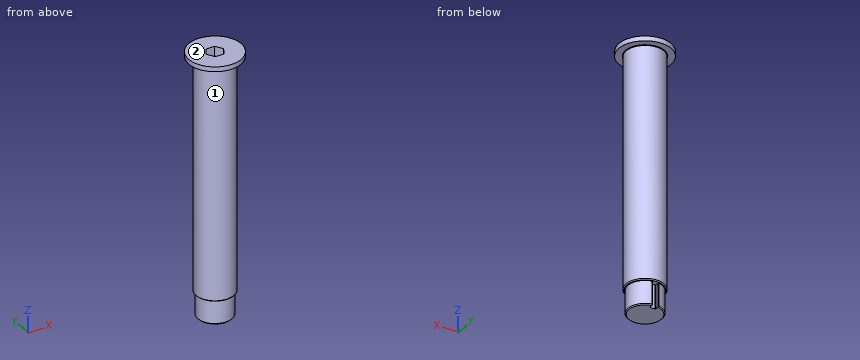
```python
from build123d import *

# Parameters (mm, degrees)
SKETCH_1_R          = 20
EXTRUDE_1_DEPTH     = 270
SKETCH_2_R          = 27.5
EXTRUDE_2_DEPTH     = 5
CUT_EXTRUDE_1_DEPTH = 10
SKETCH_4_OUTSIDE_W  = 114.158
SKETCH_4_OUTSIDE_H  = 114.158
SKETCH_4_OUTSIDE_R  = 18
CUT_EXTRUDE_2_DEPTH = 25
CHAMFER_1_SIZE      = 1
CHAMFER_2_SIZE      = 1
FILLET_1_R          = 0.5
SKETCH_5_W          = 6
SKETCH_5_H          = 10
CUT_EXTRUDE_3_DEPTH = 25
FILLET_2_R          = 0.5


with BuildPart() as part:
    # 草图1 → 凸台-拉伸1 (new body)
    with BuildSketch(Plane.XY):
        Circle(SKETCH_1_R)
    extrude(amount=EXTRUDE_1_DEPTH)

    # 草图2 → 凸台-拉伸2 (add)
    with BuildSketch(Plane.XY.offset(270)):
        Circle(SKETCH_2_R)
    extrude(amount=EXTRUDE_2_DEPTH)

    # 草图3 → 切除-拉伸1 (cut)
    with BuildSketch(Plane.XY.offset(275)):
        Polygon((9.237604307, 0), (4.618802154, 8), (-4.618802154, 8), (-9.237604307, 0), (-4.618802154, -8), (4.618802154, -8), align=None)
    extrude(amount=-CUT_EXTRUDE_1_DEPTH, mode=Mode.SUBTRACT)

    # 草图4 outside → 切除-拉伸2 (cut)
    with BuildSketch(Plane(origin=(0, 0, 0), x_dir=(-1, 0, 0), z_dir=(0, 0, -1))):
        Rectangle(SKETCH_4_OUTSIDE_W, SKETCH_4_OUTSIDE_H)
        Circle(SKETCH_4_OUTSIDE_R, mode=Mode.SUBTRACT)
    extrude(amount=-CUT_EXTRUDE_2_DEPTH, mode=Mode.SUBTRACT)

    # 倒角1
    chamfer_1_edges = [part.edges().sort_by_distance(p)[0] for p in [
        (-20, 0, 25),
    ]]
    chamfer(chamfer_1_edges, length=CHAMFER_1_SIZE)

    # 倒角2
    chamfer_2_edges = [part.edges().sort_by_distance(p)[0] for p in [
        (18, 0, 0),
    ]]
    chamfer(chamfer_2_edges, length=CHAMFER_2_SIZE)

    # 圆角1
    fillet_1_edges = [part.edges().sort_by_distance(p)[0] for p in [
        (-20, 0, 270),
    ]]
    fillet(fillet_1_edges, radius=FILLET_1_R)

    # 草图5 → 切除-拉伸3 (cut)
    with BuildSketch(Plane(origin=(0, 0, 0), x_dir=(-1, 0, 0), z_dir=(0, 0, -1))):
        with Locations((0, 18)):
            Rectangle(SKETCH_5_W, SKETCH_5_H)
    extrude(amount=-CUT_EXTRUDE_3_DEPTH, mode=Mode.SUBTRACT)

    # 圆角2
    fillet_2_edges = [part.edges().sort_by_distance(p)[0] for p in [
        (3, 13, 12.5),
        (-3, 13, 12.5),
        (-3, 17.748239349, 13),
        (3, 17.748239349, 13),
    ]]
    fillet(fillet_2_edges, radius=FILLET_2_R)


solid = part.part
```
The listing builds one solid part. Answer for the finished solid, in the listing's coordinates (mm). Face numbers are marked on the shaded views. A direction names the side the tool comes from. Give positions to 0.01 mm unless a question says otherwise; leave off trailing zeros. Order: outer loops, then holes, each group sorted by start corner. A loop starts at its lowest first (then second) coordinate and runs counter-clockwise, first axis right, second up.
Item 1: The part is cut by section B-B, the plane z = 235. Give the vertices of the cut face in (x, y), and give its area (3 significant figures).
From the geometry:
outline: circle Ø40 at (0, 0)
area: 1,260 mm2
Item 2: The part is cut by section A-A, the plane x = 0. Give the vertices of the cut face in (y, z), and give its area (3 significant figures).
From the geometry:
outline: (-27.5, 270) - (-20.5, 270) arc R0.5 cw to (-20, 269.5) - (-20, 26) - (-19, 25) - (-18, 25) - (-18, 1) - (-17, 0) - (13, 0) - (13, 25) - (19, 25) - (20, 26) - (20, 269.5) arc R0.5 cw to (20.5, 270) - (27.5, 270) - (27.5, 275) - (8, 275) - (8, 265) - (-8, 265) - (-8, 275) - (-27.5, 275) - close
area: 10,700 mm2
Item 3: Which of the six approach directions +Z, -Z, +X, -X, +Y, -Y give full straight-line access (tool end or side, diameter ignored) to the marked faces 1 and 2?
From the geometry:
face 1: -Z
face 2: +Z, +X, -X, +Y, -Y
Item 4: Given pin 1 Ø8 at (y, z) = (8, 108.5) entering from -X; pin 2 Ø3 at (x, z) = (-1.5, 270.5) entering from -Y; pin 3 Ø17.5 at (x, y) = (-2.5, -3) entering from +Z; pin 4 Ø10 at (x, z) = (16, 162.5) entering from -Y, each flat-ended and moving along its own axis, determine where each tip first touches the part or whether it passes through.
From the geometry:
pin 1: stops at x = -19.6
pin 2: stops at y = -27.5
pin 3: stops at z = 275
pin 4: stops at y = -16.7
Item 5: Find the intervals of material crossed by probe 1 along Z at (x, y) = (-20, 6); probe 2 along Y at (x, z) = (-10.5, 40); probe 3 along Z at (x, y) = (11, -15), in increasing order.
From the geometry:
probe 1: z = 270 to 275
probe 2: y = -17.02 to 17.02
probe 3: z = 25 to 275
